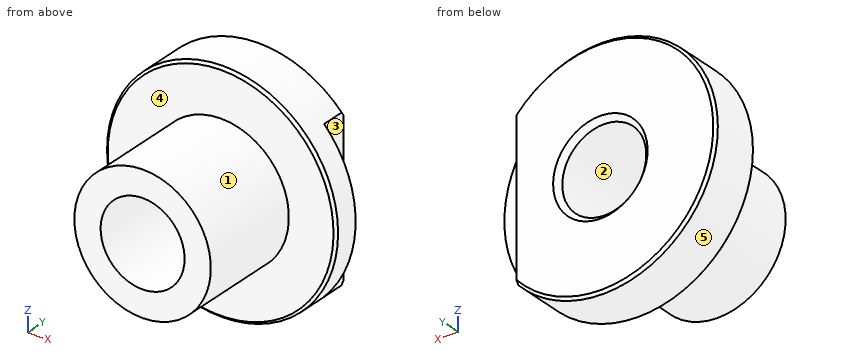
```python
from build123d import *

# Parameters (mm, degrees)
CHAMFER1_SIZE      = 0.5
CHAMFER2_SIZE      = 1
SKETCH2_W          = 20.223718868
SKETCH2_H          = 51.853895089
CUT_EXTRUDE1_DEPTH = 5


with BuildPart() as part:
    # Sketch1 → Revolve1 (revolve)
    with BuildSketch(Plane.XY, mode=Mode.PRIVATE) as revolve1_sk:
        Polygon((-22, 18.531875125), (-22, 8.531875125), (-13, 8.531875125), (-13, -11.468124875), (-8, -11.468124875), (-8, 18.531875125), align=None)
    revolve(revolve1_sk.sketch.rotate(Axis((0, 40.811378681, 0), (0, -1, 0)), 270), axis=Axis((0, 40.811378681, 0), (0, -1, 0)))

    # Chamfer1
    chamfer1_edges = [part.edges().sort_by_distance(p)[0] for p in [
        (0, 8.531875125, -22),
        (0, 18.531875125, -22),
    ]]
    chamfer(chamfer1_edges, length=CHAMFER1_SIZE)

    # Chamfer2
    chamfer2_edges = [part.edges().sort_by_distance(p)[0] for p in [
        (0, 18.531875125, -8),
    ]]
    chamfer(chamfer2_edges, length=CHAMFER2_SIZE)

    # Sketch2 → Cut-Extrude1 (cut)
    with BuildSketch(Plane(origin=(0, 18.531875125, 0), x_dir=(1, 0, 0), z_dir=(0, 1, 0))):
        with Locations((26.111859434, -0.909717457)):
            Rectangle(SKETCH2_W, SKETCH2_H)
    extrude(amount=-CUT_EXTRUDE1_DEPTH, mode=Mode.SUBTRACT)


solid = part.part
```
Build history of the part. All positions in model axes, mm. Face numbers are marked on the shaded views. A direction names the side the tool comes from. Give positions to 0.01 mm unless a question says otherwise; leave off trailing zeros. Loops run counter-clockwise (first coordinate to the right, second up) from the corner with the lowest first, then second, coordinate; pieces in that order, holes last. Notation, with made-up numbers: (28, 45.5) -> (82, 45.5) arc R18 cw to (82, 62.5) -> close; hole circle Ø2 at (-7, 85.25). An arc over 180 degrees is marked (long way). One line per question, with ' | ' between items. Start each with the question number.
1) Cut at A-A (z = 0). Give the cut face in (x, y).
2) Pin check, flat tips, straight feed: pin 1 (1.5 mm diameter, centred on y = 4.5, z = 5.5, fed in from +X); pin 2 (12 mm diameter, centred on y = 5, z = 4, fed in from -X); pin 3 (2 mm diameter, centred on y = 8.5, z = -2.5, fed in from -X). Stop position of each tip, or through.
3) Cut at B-B (x = 0). Give the cut face in (y, z), plus the area to 4 significant figures.
4) Two-plate mould, pull along Z, no slides. Class the marked faces 1, 2 and 3: released by +Z, released by -Z, zero draft, split by the parting line, or undercut.
5) Cut at C-C (y = -2). Give the cut face in (x, z).
6) Probe L1, parallel to X at y = -1, z = 0; L2, parallel to X at y = 10, z = 0; L3, parallel to Y at x = -18.5, z = 7.5. List the from-to ranges inside material, lowest first.
7) 3-axis set-ups, long thin cutter, end or side, ignore diameter. For the marked faces 4 and 5: which of +Z, -Z, +X, -X, +Y, -Y reach the whole face in a straight line?
Return value:
1) outline: (-22, 9.03) -> (-21.5, 8.53) -> (-13, 8.53) -> (-13, -11.47) -> (-8, -11.47) -> (-8, 17.53) -> (-9, 18.53) -> (-21.5, 18.53) -> (-22, 18.03) -> close; (8, -11.47) -> (13, -11.47) -> (13, 8.53) -> (21.5, 8.53) -> (22, 9.03) -> (22, 13.53) -> (16, 13.53) -> (16, 18.53) -> (9, 18.53) -> (8, 17.53) -> close
2) pin 1: x = 12.1 | pin 2: x = -22 | pin 3: x = -21.94
3) outline: (-11.47, -13) -> (8.53, -13) -> (8.53, -21.5) -> (9.03, -22) -> (18.03, -22) -> (18.53, -21.5) -> (18.53, -9) -> (17.53, -8) -> (-11.47, -8) -> close; (-11.47, 8) -> (17.53, 8) -> (18.53, 9) -> (18.53, 21.5) -> (18.03, 22) -> (9.03, 22) -> (8.53, 21.5) -> (8.53, 13) -> (-11.47, 13) -> close | area: 478.5 mm^2
4) face 1: split by the parting line | face 2: undercut | face 3: zero draft
5) outline: circle Ø26 at (0, 0); hole circle Ø16 at (0, 0)
6) L1: -13 to -8, 8 to 13 | L2: -22 to -8, 8 to 22 | L3: 8.53 to 18.53
7) face 4: -Y | face 5: +Y, -Y
